Read the model definition and answer for the solid it produces. Units are mm, in the model's axes. A direction names the side the tool comes from. Give positions to 0.01 mm unless a question says otherwise; leave off trailing zeros. Order: outer loops, then holes, each group sorted by start corner. A loop starts at its lowest first (then second) coordinate and runs counter-clockwise, first axis right, second up. Notation, with made-up numbers: (80.5, 37) -> (128.5, 37) arc R20 ccw to (128.5, 69) -> close; hole circle Ø11 at (2, 11). An arc over 180 degrees is marked (long way). Use one line per item in the form item = value.
```python
from build123d import *

# Parameters (mm, degrees)
FLANGE_PROFILE_R            = 60
FLANGE_120_DEPTH            = 35
HUB_PROFILE_R               = 30
HUB_DEPTH                   = 30
HALF_BEARING_SADDLE_DEPTH   = 60
FLANGE_RECESS_PROFILE_R     = 55
FLANGE_RECESS_110_DEPTH     = 15
FLANGE_BOLT_HOLES_PROFILE_R = 5
FLANGE_BOLT_HOLES_DEPTH     = 52
SADDLE_BORE_R20_DEPTH       = 60
SHAFT_BORE_PROFILE_R        = 12.5
SHAFT_BORE_25_DEPTH         = 60
MOUNTING_LUG_A_DEPTH        = 30
MOUNTING_LUG_B_DEPTH        = 30
LUG_BRIDGE_PROFILE_W        = 60
LUG_BRIDGE_PROFILE_H        = 32
LUG_BRIDGE_DEPTH            = 30
BRIDGE_BORE_RELIEF_DEPTH    = 35
LUG_HOLES_PROFILE_R         = 8
LUG_HOLES_2X_16_DEPTH       = 35


with BuildPart() as part:
    # Flange Profile → Flange Ø120 (new body)
    with BuildSketch(Plane.XY):
        Circle(FLANGE_PROFILE_R)
    extrude(amount=-FLANGE_120_DEPTH)

    # Hub Profile → Hub (add)
    with BuildSketch(Plane.XY):
        Circle(HUB_PROFILE_R)
    extrude(amount=HUB_DEPTH)

    # Saddle Profile → Half-Bearing Saddle (add)
    with BuildSketch(Plane.XY.offset(30)):
        with BuildLine():
            Line((-30, 0), (30, 0))
            ThreePointArc((30, 0), (0, -30), (-30, 0))
        make_face()
    extrude(amount=HALF_BEARING_SADDLE_DEPTH)

    # Flange Recess Profile → Flange Recess Ø110 (cut)
    with BuildSketch(Plane(origin=(0, 0, -35), x_dir=(-1, 0, 0), z_dir=(0, 0, -1))):
        Circle(FLANGE_RECESS_PROFILE_R)
    extrude(amount=-FLANGE_RECESS_110_DEPTH, mode=Mode.SUBTRACT)

    # Flange Bolt Holes Profile → Flange Bolt Holes (cut)
    with BuildSketch(Plane.XY):
        with Locations((45, 0)):
            Circle(FLANGE_BOLT_HOLES_PROFILE_R)
        with Locations((0, 45)):
            Circle(FLANGE_BOLT_HOLES_PROFILE_R)
        with Locations((-45, 0)):
            Circle(FLANGE_BOLT_HOLES_PROFILE_R)
        with Locations((0, -45)):
            Circle(FLANGE_BOLT_HOLES_PROFILE_R)
    extrude(amount=-FLANGE_BOLT_HOLES_DEPTH, mode=Mode.SUBTRACT)

    # Saddle Bore Profile → Saddle Bore R20 (cut)
    with BuildSketch(Plane.XY.offset(90)):
        with BuildLine():
            Line((-20, 0), (20, 0))
            ThreePointArc((20, 0), (0, -20), (-20, 0))
        make_face()
    extrude(amount=-SADDLE_BORE_R20_DEPTH, mode=Mode.SUBTRACT)

    # Shaft Bore Profile → Shaft Bore Ø25 (cut)
    with BuildSketch(Plane.XY.offset(30)):
        Circle(SHAFT_BORE_PROFILE_R)
    extrude(amount=-SHAFT_BORE_25_DEPTH, mode=Mode.SUBTRACT)



with BuildPart() as body_2:
    # Mounting Lug A Profile → Mounting Lug A (new body)
    with BuildSketch(Plane(origin=(0, 0, 0), x_dir=(1, 0, 0), z_dir=(0, 1, 0))):
        with BuildLine():
            Line((-44, -76), (-30, -76))
            Line((-30, -76), (-30, -44))
            Line((-30, -44), (-44, -44))
            ThreePointArc((-44, -44), (-60, -60), (-44, -76))
        make_face()
    extrude(amount=-MOUNTING_LUG_A_DEPTH)


with BuildPart() as body_3:
    # Mounting Lug B Profile → Mounting Lug B (new body)
    with BuildSketch(Plane(origin=(0, 0, 0), x_dir=(1, 0, 0), z_dir=(0, 1, 0))):
        with BuildLine():
            Line((44, -44), (30, -44))
            Line((30, -44), (30, -76))
            Line((30, -76), (44, -76))
            ThreePointArc((44, -76), (60, -60), (44, -44))
        make_face()
    extrude(amount=-MOUNTING_LUG_B_DEPTH)


with BuildPart() as part_1:
    add(part.part)

    add(body_2.part)  # Lug Bridge merges body 2

    add(body_3.part)  # Lug Bridge merges body 3
    # Lug Bridge Profile → Lug Bridge (add)
    with BuildSketch(Plane.XZ.offset(30)):
        with Locations((0, 60)):
            Rectangle(LUG_BRIDGE_PROFILE_W, LUG_BRIDGE_PROFILE_H)
    extrude(amount=-LUG_BRIDGE_DEPTH)

    # Bridge Relief Profile → Bridge Bore Relief (cut)
    with BuildSketch(Plane.XY.offset(76)):
        with BuildLine():
            Line((-20, 0), (20, 0))
            ThreePointArc((20, 0), (0, -20), (-20, 0))
        make_face()
    extrude(amount=-BRIDGE_BORE_RELIEF_DEPTH, mode=Mode.SUBTRACT)

    # Lug Holes Profile → Lug Holes 2xØ16 (cut)
    with BuildSketch(Plane(origin=(0, 0, 0), x_dir=(1, 0, 0), z_dir=(0, 1, 0))):
        with Locations(Location((-44, -60, 0), (0, 0, 270))):
            Circle(LUG_HOLES_PROFILE_R)
        with Locations(Location((44, -60, 0), (0, 0, 270))):
            Circle(LUG_HOLES_PROFILE_R)
    extrude(amount=-LUG_HOLES_2X_16_DEPTH, mode=Mode.SUBTRACT)


solid = part_1.part
```
Item 1: The part is cut by section C-C on x = -2. State how many separate pieces and enclosed holes the cut face has, and give its area (3 significant figures).
Checks:
separate_pieces = 4
enclosed_holes = 0
area = 3,350 mm²
Item 2: Straight lines are drawn through the part: L1, parallel to Y at x = 0, z = -15; L2, parallel to X at y = -22, z = 60; L3, parallel to Y at x = 0, z = 11. For each, find the intervals that lie inside material, in ascending order. Write a range as from..to.
Checks:
L1 = -60..-50, -40..-12.5, 12.5..40, 50..60
L2 = -60..-52, -36..36, 52..60
L3 = -30..-12.5, 12.5..30
Item 3: Given pin 1 Ø18.5 at (x, z) = (-44, 60) entering from +Y; pin 2 Ø9 at (x, y) = (-18.5, -9) entering from -Z; pin 3 Ø10 at (x, z) = (12.5, -22.5) entering from +Y; pin 4 Ø8 at (y, z) = (-30.5, 62.5) entering from +X, each flat-ended and moving along its own axis, determine where each tip first touches the part or whether it passes through.
Checks:
pin_1 = 0
pin_2 = -20
pin_3 = 59.53
pin_4 = 60
Item 4: Determine the mould class of faces 1 (the cylindrical face through (-0.651, -40.043, -9.86)), 2 (the cylindrical face through (-3.905, -29.745, 16.803)), 3 (the flat face through (-35.8, 0, 59.6)) for opening direction X: +X half, -X half, draft (parallel to the pull), parting line (faces both ways), or undercut.
Checks:
face_1 = undercut
face_2 = parting line
face_3 = draft
Item 5: Which of the six approach directions +Z, -Z, +X, -X, +Y, -Y give full straight-line access (tool end or side, diameter ignored) to faces 4 (the flat face through (-7, 11, 30)), 5 (the flat face through (-32, -19, 76)), 6 (the cylindrical face through (-50, 0, -10)), 7 (the flat face through (12, 28, 0)), 8 (the cylindrical face through (0.66, -29.993, 82.902))?
Checks:
face_4 = +Z, +Y
face_5 = +Z, -X, -Y
face_6 = -Z
face_7 = none
face_8 = +Z, -Y
Item 6: The part is cut by section B-B on y = 9.5. Give the vertices of the cut face in (x, z).
Checks:
outline = (-59.24, -35) -> (-54.17, -35) -> (-54.17, -20) -> (-8.12, -20) -> (-8.12, 30) -> (-28.46, 30) -> (-28.46, 0) -> (-59.24, 0) -> close; (8.12, -20) -> (54.17, -20) -> (54.17, -35) -> (59.24, -35) -> (59.24, 0) -> (28.46, 0) -> (28.46, 30) -> (8.12, 30) -> close
Item 7: The part is cut by section A-A on z = 60. Give the vertices of the cut face in (x, y), and give its area (3 significant figures).
Checks:
outline = (-60, -30) -> (-52, -30) -> (-52, 0) -> (-60, 0) -> close; (-36, -30) -> (36, -30) -> (36, 0) -> (20, 0) arc R20 cw to (-20, 0) -> (-36, 0) -> close; (52, -30) -> (60, -30) -> (60, 0) -> (52, 0) -> close
area = 2,010 mm²
